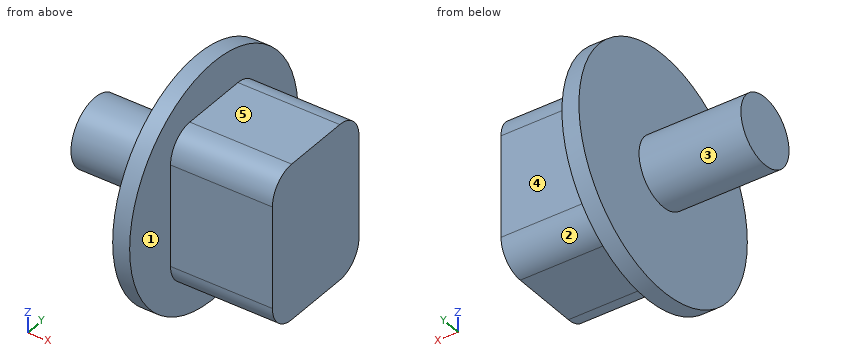
from build123d import *

# Parameters (mm, degrees)
BOSS_EXTRUDE1_DEPTH = 30


with BuildPart() as part:
    # Sketch2 → Boss-Extrude1 (new body)
    with BuildSketch(Plane(origin=(0, 0, 0), x_dir=(0, 0, -1), z_dir=(1, 0, 0))):
        with BuildLine():
            Line((-15, 18), (15, 18))
            ThreePointArc((15, 18), (20.656854249, 15.656854249), (23, 10))
            Line((23, 10), (23, -10))
            ThreePointArc((23, -10), (20.656854249, -15.656854249), (15, -18))
            Line((15, -18), (-15, -18))
            ThreePointArc((-15, -18), (-20.656854249, -15.656854249), (-23, -10))
            Line((-23, -10), (-23, 10))
            ThreePointArc((-23, 10), (-20.656854249, 15.656854249), (-15, 18))
        make_face()
    extrude(amount=-BOSS_EXTRUDE1_DEPTH)

    # Sketch3 → Revolve1 (revolve)
    with BuildSketch(Plane.XY, mode=Mode.PRIVATE) as revolve1_sk:
        Polygon((-30, 0), (-30, 35), (-35, 35), (-35, 10), (-65, 10), (-65, 0), align=None)
    revolve(revolve1_sk.sketch.rotate(Axis((-65, 0, 0), (1, 0, 0)), 180), axis=Axis((-65, 0, 0), (1, 0, 0)))


solid = part.part
Can you work these out from the model? Positions are in its coordinate system, mm. Face numbers are marked on the shaded views. A direction names the side the tool comes from. Give positions to 0.01 mm unless a question says otherwise; leave off trailing zeros. Order: outer loops, then holes, each group sorted by start corner. A loop starts at its lowest first (then second) coordinate and runs counter-clockwise, first axis right, second up. Notation, with made-up numbers: (6.5, 73.25) - (54.5, 73.25) arc R25 ccw to (54.5, 93.25) - close; hole circle Ø8 at (49, 34). An arc over 180 degrees is marked (long way). Write each question's results on one line, items separated by ' | '.
1) Suppose I cut it at A-A, the plane z = 0. Write out the boundary of the cut face in (x, y), then the cut area to 3 significant figures.
Final values:
outline: (-65, -10) - (-35, -10) - (-35, -35) - (-30, -35) - (-30, -18) - (0, -18) - (0, 18) - (-30, 18) - (-30, 35) - (-35, 35) - (-35, 10) - (-65, 10) - close | area: 2,030 mm^2
2) Suppose I cut it at D-D, the plane z = -14. Write out the boundary of the cut face in (x, y).
Final values:
outline: (-35, -32.08) - (-30, -32.08) - (-30, -18) - (0, -18) - (0, 18) - (-30, 18) - (-30, 32.08) - (-35, 32.08) - close
3) Please list where these lines run through material, in increasing order: line 1 along Y through (x, z) = (-39.5, 0.5); line 2 along X through (y, z) = (-22, 19.5); line 3 along X through (y, z) = (9.5, 20). Write a range as [from, to].
Final values:
line 1: y = [-9.99, 9.99] | line 2: x = [-35, -30] | line 3: x = [-35, 0]
4) Suppose I cut it at B-B, the plane x = -21. Write out the boundary of the cut face in (y, z), then the cut area to 3 significant figures.
Final values:
outline: (-18, -15) arc R8 ccw to (-10, -23) - (10, -23) arc R8 ccw to (18, -15) - (18, 15) arc R8 ccw to (10, 23) - (-10, 23) arc R8 ccw to (-18, 15) - close | area: 1,600 mm^2
5) On a 3-axis mill with a long thin cutter (end or side, diameter ignored), from which of +Z, -Z, +X, -X, +Y, -Y can I reach the whole of each face in a straight line? I mean the marked faces 1, 2, 3, 4 and 5. Say none if no direction works.
Final values:
face 1: +X | face 2: -Z, +X, +Y | face 3: -X | face 4: +Z, -Z, +X, +Y | face 5: +Z, +X, +Y, -Y
6) Suppose I cut it at C-C, the plane y = 0. Write out the boundary of the cut face in (x, z).
Final values:
outline: (-65, -10) - (-35, -10) - (-35, -35) - (-30, -35) - (-30, -23) - (0, -23) - (0, 23) - (-30, 23) - (-30, 35) - (-35, 35) - (-35, 10) - (-65, 10) - close
7) I'm going to push flat-ended pins straight in: pin 1 Ø3 at (x, z) = (-21.5, 19.5) entering from -Y; pin 2 Ø5 at (x, z) = (-33, 15) entering from -Y; pin 3 Ø8 at (x, z) = (-47.5, -16) entering from -Y; pin 4 Ø24 at (x, z) = (-9, -2) entering from +Y. Where does each tip first touch, or does it pass through?
Final values:
pin 1: stops at y = -17.42 | pin 2: stops at y = -32.69 | pin 3: passes through | pin 4: stops at y = 18
